```python
from build123d import *

# Parameters (mm, degrees)
FEATURE_19_WELDMEMBERFEAT_4_MORE_IN_5_DEPTH = 1420.5
CUT_EXTRUDE1_DEPTH                          = 1423.654297431
CUT_EXTRUDE1_DEPTH_BACK                     = 1423.654297431


with BuildPart() as part:
    # Sketch1 → feature 19 (WeldMemberFeat) (+4 more in 5 files) Cold-formed Hollow Structural Square Steel(gb t6728-2002) 70×70×5(1) (new body)
    with BuildSketch(Plane(origin=(0, 0, 0), x_dir=(-1, 0, 0), z_dir=(0, 1, 0))):
        with BuildLine():
            Line((-25, -35), (25, -35))
            ThreePointArc((25, -35), (32.071067812, -32.071067812), (35, -25))
            Line((35, -25), (35, 25))
            ThreePointArc((35, 25), (32.071067812, 32.071067812), (25, 35))
            Line((25, 35), (-25, 35))
            ThreePointArc((-25, 35), (-32.071067812, 32.071067812), (-35, 25))
            Line((-35, 25), (-35, -25))
            ThreePointArc((-35, -25), (-32.071067812, -32.071067812), (-25, -35))
        make_face()
        with BuildLine():
            Line((-25, -30), (25, -30))
            ThreePointArc((25, -30), (28.535533906, -28.535533906), (30, -25))
            Line((30, -25), (30, 25))
            ThreePointArc((30, 25), (28.535533906, 28.535533906), (25, 30))
            Line((25, 30), (-25, 30))
            ThreePointArc((-25, 30), (-28.535533906, 28.535533906), (-30, 25))
            Line((-30, 25), (-30, -25))
            ThreePointArc((-30, -25), (-28.535533906, -28.535533906), (-25, -30))
        make_face(mode=Mode.SUBTRACT)
    extrude(amount=FEATURE_19_WELDMEMBERFEAT_4_MORE_IN_5_DEPTH)

    # 0:feat:20/0 feature 20/0 (ProfileFeature) (+11 more in 7 files) Sketch2 → Cut-Extrude1 (cut, two sides: drawn at the far end of the back side and taken through both)
    with BuildSketch(Plane.XY.offset(35).offset(-CUT_EXTRUDE1_DEPTH_BACK)):
        Polygon((-35, 66.713584391), (35, 0), (-35, 0), align=None)
        Polygon((-35, 1420.5), (35, 1353.786415609), (35, 1420.5), align=None)
    extrude(amount=CUT_EXTRUDE1_DEPTH + CUT_EXTRUDE1_DEPTH_BACK, mode=Mode.SUBTRACT)


solid = part.part
```
For this review, take the finished solid that the model builds, in its own axes (mm). A direction names the side the tool comes from. Give positions to 0.01 mm unless a question says otherwise; leave off trailing zeros. Loops run counter-clockwise (first coordinate to the right, second up) from the corner with the lowest first, then second, coordinate; pieces in that order, holes last. Notation, with made-up numbers: M 70,87 L 92,87 A28 cw 92,108 Z; hole C 18,32.25 d3. An arc over 180 degrees is marked long. One line per item, written item: value. Start each with the question number.
Q1. Add section A-A (y = 1242). Give the boundary of the cut face in (x, z), and give its area (3 significant figures).
Q2. Add section B-B (z = -2). Give the boundary of the cut face in (x, y).
Q3. Add section C-C (x = -4). Give the boundary of the cut face in (y, z), and give its area (3 significant figures).
Q4. Machinability: for faces 4 (the face through (0, 700, -35)), 5 (the face through (0, 700, 30)), which of the approach directions +Z, -Z, +X, -X, +Y, -Y give a long, thin tool a straight path to every point of the face, cutting with its end or side? Answer none if there is none.
Q5. For L1, parallel to Z at x = -1, y = 202; L2, parallel to Z at x = 26.5, y = 1101, list the stretches that pass through material, from the lowest coordinate up.
Q6. Clearance check with a flat-ended pin moving along its axis: pin 1 Ø6 at (x, z) = (2.5, 24.5) entering from -Y. State where the tip first meets the part, or that it passes through.
Q7. Draft analysis for pull direction X (two halves, no side actions). For faces 1 (the face through (-0.49, 1387.61, 30.62)), 2 (the face through (-30, 729, 0)), 3 (the face through (0, 700, 35)), state which applies: released by +X, released by -X, zero draft, split by the parting line, or undercut.
Reply:
1. outline: M -35,-25 A10 ccw -25,-35 L 25,-35 A10 ccw 35,-25 L 35,25 A10 ccw 25,35 L -25,35 A10 ccw -35,25 Z; hole M -30,-25 A5 ccw -25,-30 L 25,-30 A5 ccw 30,-25 L 30,25 A5 ccw 25,30 L -25,30 A5 ccw -30,25 Z
1. area: 1,240 mm²
2. outline: M -35,66.71 L -30,61.95 L -30,1415.73 L -35,1420.5 Z; M 30,4.77 L 35,0 L 35,1353.79 L 30,1358.55 Z
3. outline: M 37.17,-35 L 1390.96,-35 L 1390.96,-30 L 37.17,-30 Z; M 37.17,30 L 1390.96,30 L 1390.96,35 L 37.17,35 Z
3. area: 13,500 mm²
4. face 4: -Z, +X, -X, +Y, -Y
4. face 5: +Y, -Y
5. L1: -35 to -30, 30 to 35
5. L2: -34.89 to -29.77, 29.77 to 34.89
6. pin 1: through
7. face 1: released by +X
7. face 2: undercut
7. face 3: zero draft
